Can you work these out from the model? Positions are in its coordinate system, mm. A direction names the side the tool comes from. Round coordinates to 2 decimals unless told otherwise and drop trailing zeros. Write each loop counter-clockwise with the first axis right and the second up, starting at its lowest first coordinate (ties: lowest second). Pieces come first, ordered by that corner, then holes.
Q1. I'm going to push flat-ended pins straight in: pin 1 Ø7 at (x, z) = (25, 10) entering from -Y; pin 2 Ø2.5 at (x, z) = (24, 11.5) entering from -Y. Where does each tip first touch, or does it pass through?
Q2. If we section it at A-A (z = 10): Please give me the cut outline in (x, y), plus the area to 3 significant figures.
Q3. If we section it at D-D (y = -2): Please give me the cut outline in (x, z), plus the area to 3 significant figures.
Q4. Please list where these lines run through material, in increasing order: line 1 along X through (y, z) = (-24.25, 10); line 2 along X through (y, z) = (-8, 10); line 3 along Y through (x, z) = (12.5, 7.25).
Q5. We'd pull the mould along X, two halves only. Please class faces 1 (the cylindrical face through (28.966, -20.14, 10.521)), 2 (the flat face through (50, -15, 10)), 3 (the flat face through (25, -15, 0)): +X half, -X half, draft (parallel to the pull), parting line (faces both ways), or undercut.
Q6. For faces 4 (the flat face through (25, -30, 5)), 5 (the flat face through (22, -10, 12)), which set-ups out of +Z, -Z, +X, -X, +Y, -Y let a thin tool reach every point of the face, with its end or its side?
Q7. If we section it at C-C (x = 25): Please give me the cut outline in (y, z), plus the area to 3 significant figures.
Q8. If we section it at B-B (y = -15): Please give me the cut outline in (x, z).
from build123d import *

# Parameters (mm, degrees)
SKETCH1_W           = 50
SKETCH1_H           = 30
BOSS_EXTRUDE1_DEPTH = 20
M8_TAPPED_HOLE1_D   = 6.8
M8_TAPPED_HOLE2_D   = 6.8
SKETCH6_R           = 4
CUT_EXTRUDE1_DEPTH  = 20


with BuildPart() as part:
    # Sketch1 → Boss-Extrude1 (new body)
    with BuildSketch(Plane.XY):
        with Locations((25, -15)):
            Rectangle(SKETCH1_W, SKETCH1_H)
    extrude(amount=BOSS_EXTRUDE1_DEPTH)

    # M8 Tapped Hole1 (through all)
    with Locations(Plane(origin=(0, 0, 0), x_dir=(-1, 0, 0), z_dir=(0, 0, -1))):
        with Locations((-12.5, -15), (-37.5, -15)):
            Hole(M8_TAPPED_HOLE1_D / 2)

    # M8 Tapped Hole2 (through all)
    with Locations(Plane(origin=(25, 0, 10), x_dir=(0, 0, 1), z_dir=(0, 1, 0))):
        with Locations((0, 0)):
            Hole(M8_TAPPED_HOLE2_D / 2)

    # Sketch6 → Cut-Extrude1 (cut)
    with BuildSketch(Plane.XZ.offset(30)):
        with Locations(Location((25, 10, 0), (0, 0, 270))):
            Circle(SKETCH6_R)
    extrude(amount=-CUT_EXTRUDE1_DEPTH, mode=Mode.SUBTRACT)


solid = part.part
A:
1. pin 1: stops at y = -10
1. pin 2: passes through
2. outline: (0, -30) - (21, -30) - (21, -10) - (21.6, -10) - (21.6, 0) - (0, 0) - close; (28.4, -10) - (29, -10) - (29, -30) - (50, -30) - (50, 0) - (28.4, 0) - close; hole circle Ø6.8 at (12.5, -15); hole circle Ø6.8 at (37.5, -15)
2. area: 1,200 mm2
3. outline: (0, 0) - (50, 0) - (50, 20) - (0, 20) - close; hole circle Ø6.8 at (25, 10)
3. area: 964 mm2
4. line 1: x = 0 to 21, 29 to 50
4. line 2: x = 0 to 21.6, 28.4 to 50
4. line 3: y = -30 to -18.4, -11.6 to 0
5. face 1: undercut
5. face 2: +X half
5. face 3: draft
6. face 4: +Z, -Z, +X, -X, -Y
6. face 5: -Y
7. outline: (-30, 0) - (0, 0) - (0, 6.6) - (-10, 6.6) - (-10, 6) - (-30, 6) - close; (-30, 14) - (-10, 14) - (-10, 13.4) - (0, 13.4) - (0, 20) - (-30, 20) - close
7. area: 372 mm2
8. outline: (0, 0) - (9.1, 0) - (9.1, 20) - (0, 20) - close; (15.9, 0) - (34.1, 0) - (34.1, 20) - (15.9, 20) - close; (40.9, 0) - (50, 0) - (50, 20) - (40.9, 20) - close; hole circle Ø8 at (25, 10)
